CAD build for the part. Positions are in the model's coordinates, mm. Face numbers are marked on the shaded views. A direction names the side the tool comes from. Round coordinates to 2 decimals unless told otherwise and drop trailing zeros. Order: outer loops, then holes, each group sorted by start corner. A loop starts at its lowest first (then second) coordinate and runs counter-clockwise, first axis right, second up. Notation, with made-up numbers: (-5.5, 51.25) -> (42.5, 51.25) arc R12 ccw to (42.5, 66.25) -> close; hole circle Ø6 at (-15.75, 52). An arc over 180 degrees is marked (long way). Return JSON: item names as keys, results as strings. Group by question number.
Q1. Cut at D-D (y = 0). Count the separate pieces of the cut face and the enclosed holes in it, then the cut area to 3 significant figures.
Q2. Cut at C-C (x = 34.5). Write the cut outline in (y, z).
Q3. Which spindle directions (+Z, -Z, +X, -X, +Y, -Y) get a long thin tool onto all of the face, cutting with end or side? Do the marked faces 1 and 2. Say none if no direction does.
Q4. Cut at A-A (y = 45). Write the cut outline in (x, z) (3 decimals).
Q5. Probe line 1 along Y through (x, z) = (0, 211); line 2 along Z through (x, y) = (-34, -38); line 3 along Z through (x, y) = (-11, -2.5). List the from-to ranges inside material, lowest first.
Q6. Flat gauge pins, fed straight in: pin 1 (4 mm diameter, centred on x = -34.5, z = 128, fed in from +Y); pin 2 (8 mm diameter, centred on x = 46, y = 17, fed in from -Z); pin 3 (23 mm diameter, centred on x = 0, y = 45, fed in from +Z). Where does each tip first touch, or does it go through?
Q7. Mould opens along Z. For the marked faces 3, 4, 5 and 6 say: +Z half, -Z half, draft (parallel to the pull), parting line (faces both ways), or undercut.
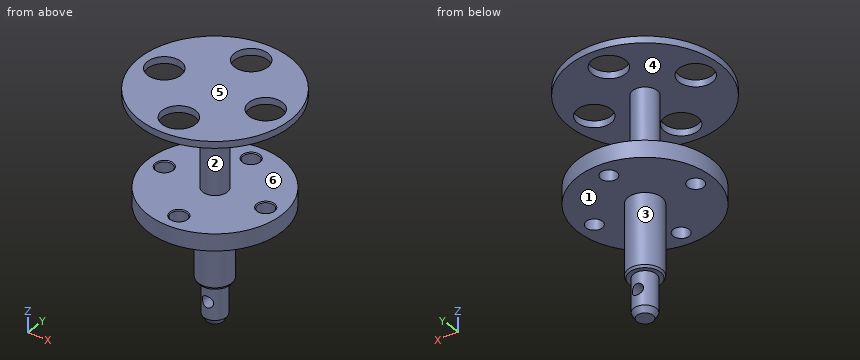
from build123d import *

# Parameters (mm, degrees)
SKETCH1_R               = 52.5
SKETCH1_R_2             = 3.5
BOSS_EXTRUDE1_DEPTH     = 14
SKETCH2_R               = 10
BOSS_EXTRUDE2_DEPTH     = 100
SKETCH3_R               = 60
BOSS_EXTRUDE3_DEPTH     = 15
CIRPATTERN1_COUNT       = 4
SKETCH6_R               = 67.698937757
CUT_EXTRUDE1_DEPTH      = 14
CHAMFER1_SIZE           = 5
CHAMFER1_SIZE2          = 2.886751346
CUT_EXTRUDE2_DEPTH      = 155.405310789
CUT_EXTRUDE2_DEPTH_BACK = 155.405310789
SKETCH7_R               = 5
SKETCH8_R               = 15
BOSS_EXTRUDE4_DEPTH     = 65
CHAMFER2_SIZE           = 2
CHAMFER2_SIZE2          = 1.154700538
SKETCH9_R               = 11
BOSS_EXTRUDE5_DEPTH     = 80
SKETCH10_R              = 67.5
SKETCH10_R_2            = 15
BOSS_EXTRUDE6_DEPTH     = 6


with BuildPart() as part:
    # Sketch1 → Boss-Extrude1 (new body)
    with BuildSketch(Plane.XY):
        Circle(SKETCH1_R)
        with Locations((0, 45)):
            Circle(SKETCH1_R_2, mode=Mode.SUBTRACT)
        with Locations((38.97114317, 22.5)):
            Circle(SKETCH1_R_2, mode=Mode.SUBTRACT)
        with Locations((38.97114317, -22.5)):
            Circle(SKETCH1_R_2, mode=Mode.SUBTRACT)
        with Locations((0, -45)):
            Circle(SKETCH1_R_2, mode=Mode.SUBTRACT)
        with Locations((-38.97114317, -22.5)):
            Circle(SKETCH1_R_2, mode=Mode.SUBTRACT)
        with Locations((-38.97114317, 22.5)):
            Circle(SKETCH1_R_2, mode=Mode.SUBTRACT)
    extrude(amount=BOSS_EXTRUDE1_DEPTH)

    # Sketch2 → Boss-Extrude2 (add)
    with BuildSketch(Plane.XY.offset(14)):
        Circle(SKETCH2_R)
    extrude(amount=BOSS_EXTRUDE2_DEPTH)

    # Sketch3 → Boss-Extrude3 (add)
    with BuildSketch(Plane.XY.offset(114)):
        Circle(SKETCH3_R)
    extrude(amount=BOSS_EXTRUDE3_DEPTH)

    # Sketch5 → M16x1.5 Tapped Hole1 (revolve, cut)
    with BuildSketch(Plane(origin=(0, 45, 129), x_dir=(0, -1, 0), z_dir=(1, 0, 0))):
        Polygon((0, 0), (0, 40.856239488), (7.25, 36.5), (7.25, 0.775), (8.025, 0), align=None)
    m16x1_5_tapped_hole1 = revolve(axis=Axis((0, 45, 135.35), (0, 0, -1)), mode=Mode.SUBTRACT)

    # CirPattern1: M16x1.5 Tapped Hole1 ×4 about axis
    cirpattern1_axis = Axis((0, 0, 0), (0, 0, 1))
    for i in range(1, CIRPATTERN1_COUNT):
        add(m16x1_5_tapped_hole1.rotate(cirpattern1_axis, i * 360 / CIRPATTERN1_COUNT), mode=Mode.SUBTRACT)

    # Sketch6 → Cut-Extrude1 (cut)
    with BuildSketch(Plane(origin=(0, 0, 0), x_dir=(-1, 0, 0), z_dir=(0, 0, -1))):
        Circle(SKETCH6_R)
    extrude(amount=-CUT_EXTRUDE1_DEPTH, mode=Mode.SUBTRACT)

    # Chamfer1
    chamfer1_edges = [part.edges().sort_by_distance(p)[0] for p in [
        (-10, 0, 14),
    ]]
    chamfer1_side = [part.faces().sort_by_distance(p)[0] for p in [
        (-10, 0, 64),
    ]]
    chamfer(chamfer1_edges, length=CHAMFER1_SIZE, length2=CHAMFER1_SIZE2, reference=chamfer1_side[0])

    # Sketch7 → Cut-Extrude2 (cut, two sides: drawn at the far end of the back side and taken through both)
    with BuildSketch(Plane(origin=(0, 0, 0), x_dir=(1, 0, 0), z_dir=(0, 1, 0)).offset(-CUT_EXTRUDE2_DEPTH_BACK)):
        with Locations(Location((0, -34, 0), (0, 0, 270))):
            Circle(SKETCH7_R)
    extrude(amount=CUT_EXTRUDE2_DEPTH + CUT_EXTRUDE2_DEPTH_BACK, mode=Mode.SUBTRACT)

    # Sketch8 → Boss-Extrude4 (add)
    with BuildSketch(Plane(origin=(0, 0, 114), x_dir=(-1, 0, 0), z_dir=(0, 0, -1))):
        with Locations(Location((0, 0, 0), (0, 0, 180))):
            Circle(SKETCH8_R)
    extrude(amount=BOSS_EXTRUDE4_DEPTH)

    # Chamfer2
    chamfer2_edges = [part.edges().sort_by_distance(p)[0] for p in [
        (-15, 0, 49),
    ]]
    chamfer2_side = [part.faces().sort_by_distance(p)[0] for p in [
        (-15, 0, 81.5),
    ]]
    chamfer(chamfer2_edges, length=CHAMFER2_SIZE, length2=CHAMFER2_SIZE2, reference=chamfer2_side[0])

    # Sketch9 → Boss-Extrude5 (add)
    with BuildSketch(Plane.XY.offset(129)):
        Circle(SKETCH9_R)
    extrude(amount=BOSS_EXTRUDE5_DEPTH)

    # Sketch10 → Boss-Extrude6 (add)
    with BuildSketch(Plane.XY.offset(209)):
        Circle(SKETCH10_R)
        with Locations((0, 45)):
            Circle(SKETCH10_R_2, mode=Mode.SUBTRACT)
        with Locations((45, 0)):
            Circle(SKETCH10_R_2, mode=Mode.SUBTRACT)
        with Locations((0, -45)):
            Circle(SKETCH10_R_2, mode=Mode.SUBTRACT)
        with Locations((-45, 0)):
            Circle(SKETCH10_R_2, mode=Mode.SUBTRACT)
    extrude(amount=BOSS_EXTRUDE6_DEPTH)


solid = part.part
Solution:
{
 "1": {"separate pieces": "5", "enclosed holes": "1", "area": "6,130 mm²"},
 "2": {"outline": "(-58.02, 209) -> (-10.71, 209) -> (-10.71, 215) -> (-58.02, 215) -> close; (-49.09, 114) -> (49.09, 114) -> (49.09, 129) -> (-49.09, 129) -> close; (10.71, 209) -> (58.02, 209) -> (58.02, 215) -> (10.71, 215) -> close"},
 "3": {"face 1": "-Z", "face 2": "none"},
 "4": {"outline": "(-50.312, 209) -> (-15, 209) -> (-15, 215) -> (-50.312, 215) -> close; (-39.686, 114) -> (-7.25, 114) -> (-7.25, 128.225) -> (-8.025, 129) -> (-39.686, 129) -> close; (7.25, 114) -> (39.686, 114) -> (39.686, 129) -> (8.025, 129) -> (7.25, 128.225) -> close; (15, 209) -> (50.312, 209) -> (50.312, 215) -> (15, 215) -> close"},
 "5": {"line 1": "y = -67.5 to -60, -30 to 30, 60 to 67.5", "line 2": "z = 114 to 129, 209 to 215", "line 3": "z = 49 to 129, 209 to 215"},
 "6": {"pin 1": "stops at y = 50.44", "pin 2": "stops at z = 114", "pin 3": "stops at z = 129"},
 "7": {"face 3": "draft", "face 4": "undercut", "face 5": "+Z half", "face 6": "undercut"}
}
